Design review of the part built by this model. Coordinates are the model's own, in mm. Give positions to 0.01 mm unless a question says otherwise; leave off trailing zeros. Write each loop counter-clockwise with the first axis right and the second up, starting at its lowest first coordinate (ties: lowest second). Pieces come first, ordered by that corner, then holes.
```python
from build123d import *

# Parameters (mm, degrees)
SKETCH1_R           = 7
SKETCH1_R_2         = 57
BOSS_EXTRUDE1_DEPTH = 1


with BuildPart() as part:
    # Sketch1 → Boss-Extrude1 (new body)
    with BuildSketch(Plane(origin=(0, 0, 0), x_dir=(1, 0, 0), z_dir=(0, 1, 0))):
        with BuildLine():
            ThreePointArc((-18.703646406, 82.916666667), (0, -85), (18.703646406, 82.916666667))
            ThreePointArc((18.703646406, 82.916666667), (0, 70), (-18.703646406, 82.916666667))
        make_face()
        with Locations(Location((-35, 60.621778265, 0), (0, 0, 270))):
            Circle(SKETCH1_R, mode=Mode.SUBTRACT)
        with Locations(Location((35, 60.621778265, 0), (0, 0, 270))):
            Circle(SKETCH1_R, mode=Mode.SUBTRACT)
        with Locations(Location((70, 0, 0), (0, 0, 270))):
            Circle(SKETCH1_R, mode=Mode.SUBTRACT)
        with Locations(Location((35, -60.621778265, 0), (0, 0, 270))):
            Circle(SKETCH1_R, mode=Mode.SUBTRACT)
        with Locations(Location((-35, -60.621778265, 0), (0, 0, 270))):
            Circle(SKETCH1_R, mode=Mode.SUBTRACT)
        with Locations(Location((-70, 0, 0), (0, 0, 270))):
            Circle(SKETCH1_R, mode=Mode.SUBTRACT)
        with Locations(Location((0, 0, 0), (0, 0, 270))):
            Circle(SKETCH1_R_2, mode=Mode.SUBTRACT)
    extrude(amount=BOSS_EXTRUDE1_DEPTH)


solid = part.part
```
(1) Consider section A-A, the plane x = 0. Give the boundary of the cut face in (y, z).
Resolved:
outline: (0, -70) - (1, -70) - (1, -57) - (0, -57) - close; (0, 57) - (1, 57) - (1, 85) - (0, 85) - close
(2) Consider section B-B, the plane z = 0. Give the boundary of the cut face in (x, y).
Resolved:
outline: (-85, 0) - (-77, 0) - (-77, 1) - (-85, 1) - close; (-63, 0) - (-57, 0) - (-57, 1) - (-63, 1) - close; (57, 0) - (63, 0) - (63, 1) - (57, 1) - close; (77, 0) - (85, 0) - (85, 1) - (77, 1) - close
(3) Consider section D-D, the plane z = -30.5. Give the boundary of the cut face in (x, y).
Resolved:
outline: (-79.34, 0) - (-48.15, 0) - (-48.15, 1) - (-79.34, 1) - close; (48.15, 0) - (79.34, 0) - (79.34, 1) - (48.15, 1) - close
(4) Consider section C-C, the plane y = 0.35. Give the boundary of the cut face in (x, z).
Resolved:
outline: (-18.7, -82.92) arc R20 cw to (18.7, -82.92) arc R85 ccw (long way) to start; hole circle Ø14 at (-70, 0); hole circle Ø114 at (0, 0); hole circle Ø14 at (-35, -60.62); hole circle Ø14 at (-35, 60.62); hole circle Ø14 at (35, -60.62); hole circle Ø14 at (35, 60.62); hole circle Ø14 at (70, 0)
(5) Mouldability with a two-part tool opening along X and no side actions: class faces 1 (the face through (-30.27, 0.49, -65.78)), 2 (the face through (18, 1, 56)), 3 (the face through (-3.47, 0.49, 84.93)) as pulls with the +X half, pulls with the -X half, needs draft (parallel to the pull), parting line crosses it, or undercut.
Resolved:
face 1: undercut
face 2: needs draft
face 3: parting line crosses it
(6) To check wall thickness, follow L1, parallel to X at y = 0.35, z = 0; L2, parallel to X at y = 0.55, z = -58.5; L3, parallel to X at y = 0.15, z = 62. State the ranges of each line that lie inside material, in increasing order.
Resolved:
L1: x = -85 to -77, -63 to -57, 57 to 63, 77 to 85
L2: x = -61.67 to -41.67, -28.33 to 28.33, 41.67 to 61.67
L3: x = -58.15 to -41.86, -28.14 to 28.14, 41.86 to 58.15
